```python
from build123d import *

# Parameters (mm, degrees)
SKETCH1_W           = 2
SKETCH1_H           = 20
BOSS_EXTRUDE1_DEPTH = 130
SKETCH2_W           = 10
SKETCH2_H           = 20
BOSS_EXTRUDE2_DEPTH = 2
SKETCH3_R           = 1.5
CUT_EXTRUDE1_DEPTH  = 6
SKETCH5_R           = 1.5
CUT_EXTRUDE2_DEPTH  = 45


with BuildPart() as part:
    # Sketch1 → Boss-Extrude1 (new body)
    with BuildSketch(Plane.XY):
        with Locations((11, 0)):
            Rectangle(SKETCH1_W, SKETCH1_H)
    extrude(amount=BOSS_EXTRUDE1_DEPTH)

    # Sketch2 → Boss-Extrude2 (add)
    with BuildSketch(Plane.XY):
        with Locations((17, 0)):
            Rectangle(SKETCH2_W, SKETCH2_H)
    extrude(amount=BOSS_EXTRUDE2_DEPTH)

    # Sketch3 → Cut-Extrude1 (cut)
    with BuildSketch(Plane.XY.offset(2)):
        with Locations((17, 5)):
            Circle(SKETCH3_R)
        with Locations((17, -5)):
            Circle(SKETCH3_R)
    extrude(amount=-CUT_EXTRUDE1_DEPTH, mode=Mode.SUBTRACT)

    # Sketch5 → Cut-Extrude2 (cut)
    with BuildSketch(Plane(origin=(12, 0, 0), x_dir=(0, 0, -1), z_dir=(1, 0, 0))):
        with Locations((-105.442155364, -5)):
            Circle(SKETCH5_R)
        with Locations((-105.442155364, 5)):
            Circle(SKETCH5_R)
    extrude(amount=-CUT_EXTRUDE2_DEPTH, mode=Mode.SUBTRACT)


solid = part.part
```
Can you work these out from the model? Positions are in its coordinate system, mm. A direction names the side the tool comes from. Round coordinates to 2 decimals unless told otherwise and drop trailing zeros. Loops run counter-clockwise (first coordinate to the right, second up) from the corner with the lowest first, then second, coordinate; pieces in that order, holes last. Notation, with made-up numbers: M -28,40.25 L -10,40.25 A25 ccw -10,74.25 Z; hole C 30,-8.5 d5. An arc over 180 degrees is marked long. Answer in a Markdown table with one row per item.
1. Please list where these lines run through material, in increasing order: line 1 (Y direction, x = 17, z = 0.75); line 2 (Z direction, x = 13.25, y = -4.5); line 3 (X direction, y = 7.75, z = 111.5). Write a range as from..to.
Established:
| item | result |
|---|---|
| line 1 | -10..-6.5, -3.5..3.5, 6.5..10 |
| line 2 | 0..2 |
| line 3 | 10..12 |
2. If we section it at C-C, the plane z = 15: Please give me the cut outline in (x, y), plus the area to 3 significant figures.
Established:
| item | result |
|---|---|
| outline | M 10,-10 L 12,-10 L 12,10 L 10,10 Z |
| area | 40.0 mm² |
3. On a 3-axis mill with a long thin cutter (end or side, diameter ignored), from which of +Z, -Z, +X, -X, +Y, -Y can I reach the whole of each face in a straight line? I mean faces 4 (the face through (11, -10, 65)), 5 (the face through (17, 0, 2)). Say none if no direction works.
Established:
| item | result |
|---|---|
| face 4 | +Z, -Z, +X, -X, -Y |
| face 5 | +Z, +X, +Y, -Y |
4. If we section it at B-B, the plane x = 14: Please give me the cut outline in (y, z).
Established:
| item | result |
|---|---|
| outline | M -10,0 L 10,0 L 10,2 L -10,2 Z |
5. If we section it at A-A, the plane y = 5: Please give me the cut outline in (x, z), plus the area to 3 significant figures.
Established:
| item | result |
|---|---|
| outline | M 10,0 L 15.5,0 L 15.5,2 L 12,2 L 12,103.94 L 10,103.94 Z; M 10,106.94 L 12,106.94 L 12,130 L 10,130 Z; M 18.5,0 L 22,0 L 22,2 L 18.5,2 Z |
| area | 268 mm² |
6. I'm going to push flat-ended pins straight in: pin 1 Ø5 at (x, y) = (15.5, 2) entering from +Z; pin 2 Ø2.5 at (y, z) = (5, 105.44) entering from +X; pin 3 Ø3 at (y, z) = (-1.5, 98.5) entering from +X. Where does each tip first touch, or does it pass through?
Established:
| item | result |
|---|---|
| pin 1 | z = 2 |
| pin 2 | through |
| pin 3 | x = 12 |
7. If we section it at D-D, the plane y = -1.75: Please give me the cut outline in (x, z).
Established:
| item | result |
|---|---|
| outline | M 10,0 L 22,0 L 22,2 L 12,2 L 12,130 L 10,130 Z |
8. Thinking about a two-plate mould opening in Z: for faces 1 (the face through (11, 0, 130)), 2 (the face through (11.01, -4.93, 106.94)), 3 (the face through (10, 0, 64)), which applies, pulls with the +Z half, pulls with the -Z half, needs draft (parallel to the pull), parting line crosses it, or undercut?
Established:
| item | result |
|---|---|
| face 1 | pulls with the +Z half |
| face 2 | undercut |
| face 3 | needs draft |
